Can you work these out from the model? Positions are in its coordinate system, mm. A direction names the side the tool comes from. Give positions to 0.01 mm unless a question says otherwise; leave off trailing zeros. Order: outer loops, then holes, each group sorted by start corner. A loop starts at its lowest first (then second) coordinate and runs counter-clockwise, first axis right, second up. Notation, with made-up numbers: M 31.25,-24 L 49.25,-24 A30 cw 49.25,4 Z; hole C 73,50.25 d8. An arc over 180 degrees is marked long. One line per question, with ' | ' between items. Start each with the question number.
1) If we section it at A-A, the plane z = 0.25: Please give me the cut outline in (x, y).
2) Thinking about a two-plate mould opening in Y: for faces 1 (the flat face through (41, 0, 0)), 2 (the flat face through (53, 34, -5)), 3 (the cylindrical face through (92.932, 54.638, -0.07)), which applies, +Y half, -Y half, draft (parallel to the pull), parting line (faces both ways), or undercut?
3) If we section it at B-B, the plane x = 83: Please give me the cut outline in (y, z), plus the area to 3 significant figures.
4) For faces 4 (the flat face through (80, 15, 0)), 5 (the flat face through (53, 34, 5)), which set-ups out of +Z, -Z, +X, -X, +Y, -Y let a thin tool reach every point of the face, with its end or its side?
5) If we section it at D-D, the plane y = 10.5: Please give me the cut outline in (x, z), plus the area to 3 significant figures.
6) If we section it at C-C, the plane y = 70: Please give me the cut outline in (x, z).
7) Please list where these lines run through material, in increasing order: line 1 along X through (y, z) = (21, 2.75); line 2 along Y through (x, z) = (84.5, -0.5); line 3 along X through (y, z) = (44.5, -1.5). Write a range as [from, to].
8) I'm going to push flat-ended pins straight in: pin 1 Ø1.5 at (y, z) = (48.5, -4) entering from -X; pin 2 Ø10 at (x, y) = (72, 58) entering from +Z; pin 3 Ø4 at (x, z) = (81.5, 3) entering from +Y. Where does each tip first touch, or does it pass through?
```python
from build123d import *

# Parameters (mm, degrees)
SKETCH1_R           = 14
BOSS_EXTRUDE1_DEPTH = 5


with BuildPart() as part:
    # Sketch1 → Boss-Extrude1 (new, symmetric)
    with BuildSketch(Plane.XY):
        with BuildLine():
            Line((0, 0), (0, 40))
            Line((0, 40), (66.869031748, 81.273873008))
            ThreePointArc((66.869031748, 81.273873008), (101.056415799, 73.476919296), (93.81926996, 39.166666667))
            Line((93.81926996, 39.166666667), (80, 30))
            Line((80, 30), (80, 0))
            Line((80, 0), (0, 0))
        make_face()
        with Locations((80, 60)):
            Circle(SKETCH1_R, mode=Mode.SUBTRACT)
    extrude(amount=BOSS_EXTRUDE1_DEPTH, both=True)


solid = part.part
```
Results found:
1) outline: M 0,0 L 80,0 L 80,30 L 93.82,39.17 A25 ccw 66.87,81.27 L 0,40 Z; hole C 80,60 d28
2) face 1: -Y half | face 2: draft | face 3: undercut
3) outline: M 31.99,-5 L 46.33,-5 L 46.33,5 L 31.99,5 Z; M 73.67,-5 L 84.82,-5 L 84.82,5 L 73.67,5 Z | area: 255 mm²
4) face 4: +Z, -Z, +X, -Y | face 5: +Z, +X, -X, +Y, -Y
5) outline: M 0,-5 L 80,-5 L 80,5 L 0,5 Z | area: 800 mm²
6) outline: M 48.6,-5 L 70.2,-5 L 70.2,5 L 48.6,5 Z; M 89.8,-5 L 102.91,-5 L 102.91,5 L 89.8,5 Z
7) line 1: x = [0, 80] | line 2: y = [32.98, 46.74], [73.26, 84.59] | line 3: x = [7.29, 99.62]
8) pin 1: stops at x = 12.56 | pin 2: passes through | pin 3: stops at y = 85
